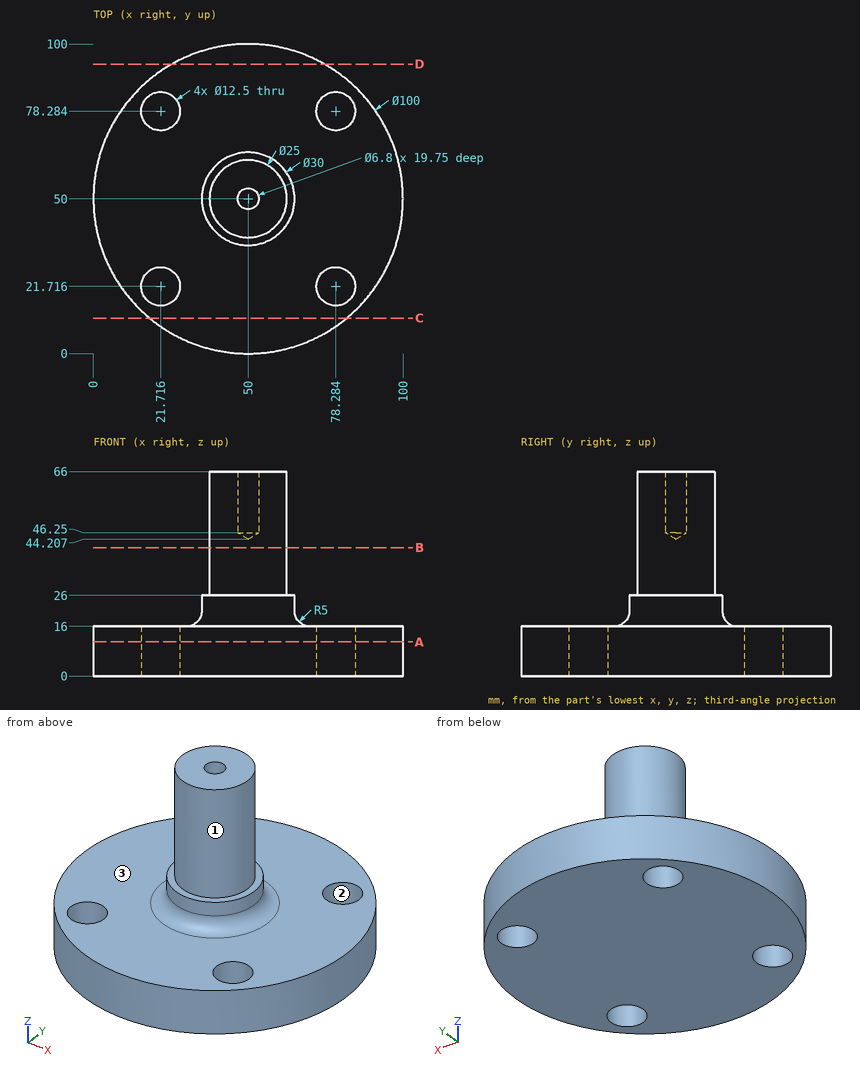
Verification items for this drawing (mm, ordinates from the low corner). Round coordinates to 2 decimals unless told otherwise and drop trailing zeros. Order: outer loops, then holes, each group sorted by start corner. A loop starts at its lowest first (then second) coordinate and runs counter-clockwise, first axis right, second up. Notation, with made-up numbers: (13, 22) -> (42, 22) arc R34 cw to (42, 61) -> close; hole circle Ø1 at (-1.5, 5.25). An arc over 180 degrees is marked (long way). Use one line per item in the form item = value.
1. Cross-section at B-B, the plane z = 41.5. Enter the section's corners in (x, y).
Working result:
outline = circle Ø25 at (50, 50)
2. Go/stop test with flat-tipped pins: pin 1 (20 mm diameter, centred on x = 21.72, y = 78.28, fed in from +Z); pin 2 (12 mm diameter, centred on y = 81, z = 9, fed in from -X); pin 3 (10 mm diameter, centred on x = 30.5, y = 22, fed in from -Z); pin 4 (10 mm diameter, centred on x = 61, z = 24, fed in from +Y). Record where each tip stops, or that it passes through.
Working result:
pin_1 = 16
pin_2 = 6.7
pin_3 = 0
pin_4 = 63.75
3. Cross-section at C-C, the plane y = 11.5. Enter the section's corners in (x, z), plus the area to 3 significant figures.
Working result:
outline = (18.1, 0) -> (81.9, 0) -> (81.9, 16) -> (18.1, 16) -> close
area = 1,020 mm^2
4. Scan lines: line 1 along Y through (x, z) = (50, 52.75); line 2 along Z through (x, y) = (39.5, 12); line 3 along Y through (x, z) = (5, 15) (1 decimal). Record each from-to range of solid material in increasing order. Write a range as from..to.
Working result:
line_1 = 37.5..46.6, 53.4..62.5
line_2 = 0..16
line_3 = 28.2..71.8
5. Mould release check, pull along X, two halves, no side actions. Record for the marked faces 1, 2 and 3: pulls with the +X half, pulls with the -X half, needs draft (parallel to the pull), parting line crosses it, or undercut.
Working result:
face_1 = parting line crosses it
face_2 = undercut
face_3 = needs draft
6. Cross-section at A-A, the plane z = 11. Enter the section's corners in (x, y).
Working result:
outline = circle Ø100 at (50, 50); hole circle Ø12.5 at (21.72, 21.72); hole circle Ø12.5 at (21.72, 78.28); hole circle Ø12.5 at (78.28, 21.72); hole circle Ø12.5 at (78.28, 78.28)
7. Cross-section at D-D, the plane y = 93.5. Enter the section's corners in (x, z).
Working result:
outline = (25.35, 0) -> (74.65, 0) -> (74.65, 16) -> (25.35, 16) -> close
